The drawing under review shows one solid part. Ordinate dimensions are in mm from its lowest x, y, z. A direction names the side the tool comes from. Round coordinates to 2 decimals unless told otherwise and drop trailing zeros. Order: outer loops, then holes, each group sorted by start corner. A loop starts at its lowest first (then second) coordinate and runs counter-clockwise, first axis right, second up. Notation, with made-up numbers: M 22,-24 L 39,-24 A20 cw 39,-13 Z; hole C -32.5,-20.75 d1. An arc over 180 degrees is marked long. Use a Markdown table: item, result.
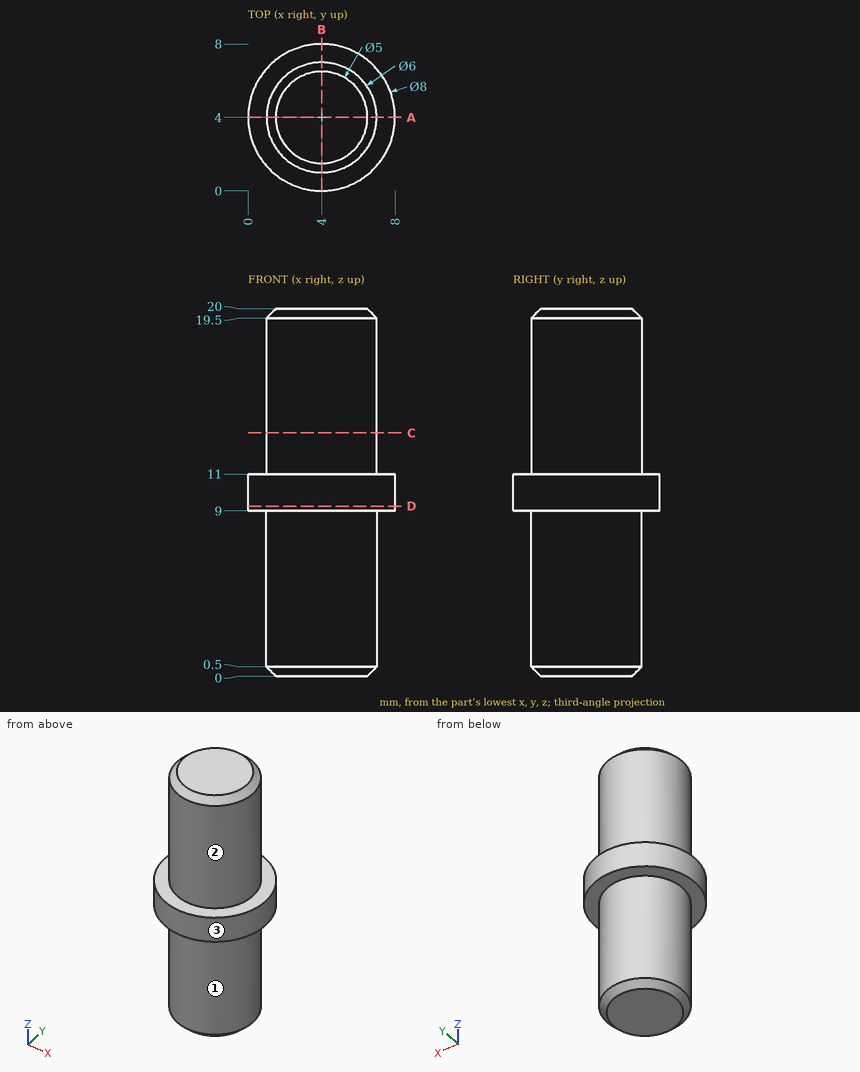
Q1. Add section D-D (z = 9.25). Write out the cut boundary in (x, y), then the cut area to 3 significant figures.
Determined:
| item | result |
|---|---|
| outline | C 4,4 d8 |
| area | 50.3 mm^2 |
Q2. Add section C-C (z = 13.25). Write out the cut boundary in (x, y), then the cut area to 3 significant figures.
Determined:
| item | result |
|---|---|
| outline | C 4,4 d6 |
| area | 28.3 mm^2 |
Q3. Wall thickness on line 1 along Z through (x, y) = (4.25, 0.75); line 2 along Y through (x, z) = (4, 8); line 3 along Y through (x, z) = (5.75, 4.5): over which ranges is each line inside the solid? List them lowest first. Write a range as [from, to].
Determined:
| item | result |
|---|---|
| line 1 | z = [9, 11] |
| line 2 | y = [1, 7] |
| line 3 | y = [1.56, 6.44] |
Q4. Add section A-A (y = 4). Write out the cut boundary in (x, z).
Determined:
| item | result |
|---|---|
| outline | M 0,9 L 1,9 L 1,0.5 L 1.5,0 L 6.5,0 L 7,0.5 L 7,9 L 8,9 L 8,11 L 7,11 L 7,19.5 L 6.5,20 L 1.5,20 L 1,19.5 L 1,11 L 0,11 Z |
Q5. Clearance check with flat-ended pins moving along their axes: pin 1 (1 mm diameter, centred on x = 6.5, z = 10.5, fed in from +Y); pin 2 (2 mm diameter, centred on x = 7, z = 5, fed in from +Y). State where each tip first meets the part, or that it passes through.
Determined:
| item | result |
|---|---|
| pin 1 | stops at y = 7.46 |
| pin 2 | stops at y = 6.24 |
Q6. Machinability: for the marked faces 1, 2 and 3, which of the approach directions +Z, -Z, +X, -X, +Y, -Y give a long, thin tool a straight path to every point of the face, cutting with its end or side? Answer none if there is none.
Determined:
| item | result |
|---|---|
| face 1 | -Z |
| face 2 | +Z |
| face 3 | +Z, -Z |
